Source: CAD feature listing. Evaluate the final solid. Frame: model axes, mm. Face numbers are marked on the shaded views. A direction names the side the tool comes from. Coordinates: 2 decimals unless noted, no trailing zeros. Loops run counter-clockwise (first coordinate to the right, second up) from the corner with the lowest first, then second, coordinate; pieces in that order, holes last. Notation, with made-up numbers: (72, 79) -> (126, 79) arc R18 ccw to (126, 93) -> close; hole circle Ø2 at (49, 42). An arc over 180 degrees is marked (long way). Answer as a JSON object with one key per item and string values. Group by question number.
from build123d import *

# Parameters (mm, degrees)
EXTRUDE_1_DEPTH     = 3.45
CHAMFER_1_SIZE      = 0.5
SKETCH_2_W          = 5.5
SKETCH_2_H          = 4.3
CUT_EXTRUDE_1_DEPTH = 19.061146143
SKETCH_3_W          = 8.7
SKETCH_3_H          = 5.5
CUT_EXTRUDE_2_DEPTH = 2.7
SKETCH_5_W          = 6.7
SKETCH_5_H          = 5.5
CUT_EXTRUDE_3_DEPTH = 14
SKETCH_6_W          = 1.1
SKETCH_6_H          = 7.4
CUT_EXTRUDE_4_DEPTH = 1
EXTRUDE_2_DEPTH     = 1.6
SKETCH_8_W          = 2
SKETCH_8_H          = 1
CUT_EXTRUDE_5_DEPTH = 3.5
SKETCH_9_R          = 0.75
EXTRUDE_3_DEPTH     = 3.2
DRAFT_1_ANGLE       = 2
CUT_EXTRUDE_6_DEPTH = 3.2
EXTRUDE_4_DEPTH     = 0.5
SCALE_1_SCALE       = 0.7


with BuildPart() as part:
    # 草图1 → 凸台-拉伸1 (new, symmetric)
    with BuildSketch(Plane.XY):
        Polygon((-3.95, 0), (3.95, 0), (3.95, 12.3), (5.5, 12.3), (5.5, 15), (-5.5, 15), (-5.5, 12.3), (-3.95, 12.3), align=None)
    extrude(amount=EXTRUDE_1_DEPTH, both=True)

    # 倒角1
    chamfer_1_edges = [part.edges().sort_by_distance(p)[0] for p in [
        (3.95, 0, 0),
        (-3.95, 0, 0),
        (0, 0, 3.45),
        (0, 0, -3.45),
    ]]
    chamfer(chamfer_1_edges, length=CHAMFER_1_SIZE)

    # 草图2 → 切除-拉伸1 (cut, through all)
    with BuildSketch(Plane.ZY.offset(3.95)):
        with Locations((0, 10.15)):
            Rectangle(SKETCH_2_W, SKETCH_2_H)
    extrude(amount=-CUT_EXTRUDE_1_DEPTH, mode=Mode.SUBTRACT)

    # 草图3 → 切除-拉伸2 (cut)
    with BuildSketch(Plane(origin=(0, 15, 0), x_dir=(1, 0, 0), z_dir=(0, 1, 0))):
        Rectangle(SKETCH_3_W, SKETCH_3_H)
    extrude(amount=-CUT_EXTRUDE_2_DEPTH, mode=Mode.SUBTRACT)

    # 草图5 → 切除-拉伸3 (cut)
    with BuildSketch(Plane(origin=(0, 15, 0), x_dir=(1, 0, 0), z_dir=(0, 1, 0))):
        Rectangle(SKETCH_5_W, SKETCH_5_H)
    extrude(amount=-CUT_EXTRUDE_3_DEPTH, mode=Mode.SUBTRACT)

    # 草图6 → 切除-拉伸4 (cut)
    with BuildSketch(Plane.XY.offset(3.45)):
        with Locations((0, 8.1)):
            Rectangle(SKETCH_6_W, SKETCH_6_H)
    extrude(amount=-CUT_EXTRUDE_4_DEPTH, mode=Mode.SUBTRACT)

    # 草图7 → 凸台-拉伸2 (add, symmetric)
    with BuildSketch(Plane.XY):
        Polygon((-3.95, 8), (-4.625, 10.1), (-4.025, 10.1), (-3.35, 8), align=None)
        Polygon((3.35, 8), (3.95, 8), (4.625, 10.1), (4.025, 10.1), align=None)
    extrude(amount=EXTRUDE_2_DEPTH, both=True)

    # 草图8 → 切除-拉伸5 (cut)
    with BuildSketch(Plane.XZ):
        with Locations((-1.55, -1.75)):
            Rectangle(SKETCH_8_W, SKETCH_8_H)
        with Locations((1.55, -1.75)):
            Rectangle(SKETCH_8_W, SKETCH_8_H)
    extrude(amount=-CUT_EXTRUDE_5_DEPTH, mode=Mode.SUBTRACT)

    # 草图9 → 凸台-拉伸3 (add)
    with BuildSketch(Plane(origin=(0, 1, 0), x_dir=(1, 0, 0), z_dir=(0, 1, 0))):
        with Locations(Location((0, -0.55, 0), (0, 0, 270))):
            Circle(SKETCH_9_R)
    extrude(amount=EXTRUDE_3_DEPTH)

    # 拔模1
    draft_1_faces = [part.faces().sort_by_distance(p)[0] for p in [
        (0, 2.6, -0.2),
    ]]
    draft(draft_1_faces, Plane.ZX.offset(1), DRAFT_1_ANGLE)

    # 草图10 → 切除-拉伸6 (cut)
    with BuildSketch(Plane(origin=(0, 0, -3.45), x_dir=(-1, 0, 0), z_dir=(0, 0, -1))):
        Polygon((-2.05, 4.3), (-2.05, 2.7), (-1.15, 3.1), (-0.2, 2.4), (1.05, 2.4), (2.05, 4.3), (2.05, 7.2), (0.15, 4), (-0.55, 4.6), align=None)
    extrude(amount=-CUT_EXTRUDE_6_DEPTH, mode=Mode.SUBTRACT)

    # 草图11 → 凸台-拉伸4 (add)
    with BuildSketch(Plane.XY.offset(-2.75)):
        Polygon((0.55, 4.6), (2.05, 4.3), (-2.05, 7.2), (-0.15, 4), align=None)
    extrude(amount=EXTRUDE_4_DEPTH)


with BuildPart() as part_1:
    # 缩放比例1: scaled about (0.005424554, 7.149122165, 0.023385792)
    add(part.part.scale(SCALE_1_SCALE).moved(Location((0.001627366, 2.14473665, 0.007015738))))


solid = part_1.part
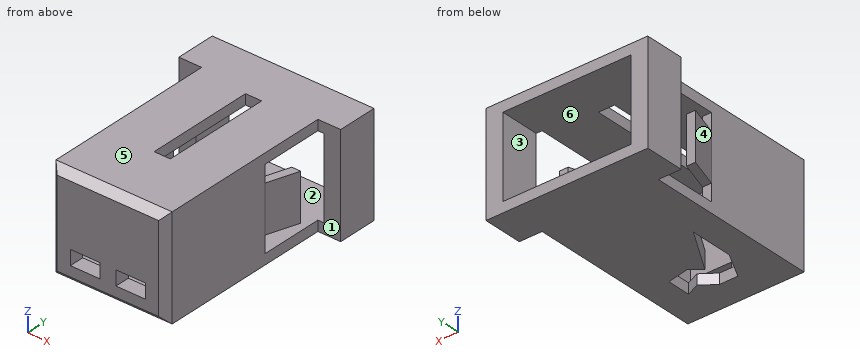
1. Section query C-C on z = -0.5. Return loops of the section in (x, y).
2. Mould query, pull axis X, two halves, no side actions, for the marked faces 1, 2, 3 and 4. Classes: pulls with the +X half, pulls with the -X half, needs draft (parallel to the pull), parting line crosses it, or undercut.
3. Section query D-D on y = 5.75. Return loops of the section in (x, z).
4. Ray query, L1, parallel to X at y = 4.5, z = 0.25; L2, parallel to X at y = 7.5, z = 1.1; L3, parallel to X at y = 6.25, z = 2.15. Return the intervals inside material, ascending.
5. Section query A-A on z = -1.8. Return loops of the section in (x, y), then the cut area to 3 significant figures.
6. Reachability of the marked faces 5 and 6 from +Z, -Z, +X, -X, +Y, -Y: full face, straight path, thin tool, end or side. Return the list, or none.
7. Pin query (flat end, axial travel): pin 1 Ø2 at (y, z) = (9.5, -2) entering from -X; pin 2 Ø1.1 at (x, y) = (0, 6.5) entering from +Z; pin 3 Ø0.5 at (y, z) = (8.5, 2) entering from +X. Return the tip coordinate at first contact, or that it passes through.
8. Section query B-B on y = 3. Return loops of the section in (x, z).
Solved:
{
 "1": {"outline": "(-3.85, 10.75) -> (-3.04, 10.75) -> (-3.04, 12.64) -> (-3.85, 12.64) -> close; (-3.24, 9.21) -> (-2.76, 7.74) -> (-2.76, 2.49) -> (-2.41, 2.14) -> (2.42, 2.14) -> (2.77, 2.49) -> (2.77, 7.74) -> (3.24, 9.21) -> (2.82, 9.21) -> (2.35, 7.74) -> (2.35, 2.84) -> (-2.34, 2.84) -> (-2.34, 7.74) -> (-2.82, 9.21) -> close; (3.05, 10.75) -> (3.85, 10.75) -> (3.85, 12.64) -> (3.05, 12.64) -> close"},
 "2": {"face 1": "needs draft", "face 2": "undercut", "face 3": "undercut", "face 4": "pulls with the -X half"},
 "3": {"outline": "(-2.76, -2.41) -> (-1.43, -2.41) -> (-1.43, -1.92) -> (-2.34, -1.92) -> (-2.34, 1.93) -> (-0.38, 1.93) -> (-0.38, 2.42) -> (-2.76, 2.42) -> close; (-0.58, -2.41) -> (2.77, -2.41) -> (2.77, 2.42) -> (0.39, 2.42) -> (0.39, 1.93) -> (2.35, 1.93) -> (2.35, -1.92) -> (0.6, -1.92) -> (0.6, -1.57) -> (-0.58, -1.57) -> close"},
 "4": {"L1": "-2.76 to -2.34, -0.44 to 0.45, 2.35 to 2.77", "L2": "-2.76 to -2.34, 2.35 to 2.77", "L3": "-2.76 to -0.38, 0.39 to 2.77"},
 "5": {"outline": "(-3.85, 10.75) -> (-3.04, 10.75) -> (-3.04, 12.64) -> (-3.85, 12.64) -> close; (-2.76, 2.49) -> (-2.41, 2.14) -> (2.42, 2.14) -> (2.77, 2.49) -> (2.77, 7.74) -> (2.35, 7.74) -> (2.35, 2.84) -> (-2.34, 2.84) -> (-2.34, 7.74) -> (-2.76, 7.74) -> close; (-1.43, 7.18) -> (-0.1, 4.94) -> (0.39, 5.36) -> (1.44, 5.15) -> close; (3.05, 10.75) -> (3.85, 10.75) -> (3.85, 12.64) -> (3.05, 12.64) -> close", "area": "12.5 mm^2"},
 "6": {"face 5": "+Z, +X, -X, +Y, -Y", "face 6": "+Y"},
 "7": {"pin 1": "x = -3.24", "pin 2": "z = 2.42", "pin 3": "x = 2.77"},
 "8": {"outline": "(-2.76, -2.41) -> (2.77, -2.41) -> (2.77, 2.42) -> (-2.76, 2.42) -> close; circle Ø1.04 at (0, 0.39); hole (-2.34, -1.92) -> (2.35, -1.92) -> (2.35, 1.93) -> (-2.34, 1.93) -> close"}
}
